Build history of the part. All positions in model axes, mm. A direction names the side the tool comes from. Round coordinates to 2 decimals unless told otherwise and drop trailing zeros. Write each loop counter-clockwise with the first axis right and the second up, starting at its lowest first coordinate (ties: lowest second). Pieces come first, ordered by that corner, then holes.
Item 1: Band-saw the part on B-B, the plane x = 65.5. Write the cut outline in (y, z) (3 decimals), then the cut area to 3 significant figures.
Item 2: Wall check: probe 1 along Y at (x, z) = (21, 83.5); probe 2 along X at (y, z) = (45.5, -12); probe 3 along Y at (x, z) = (14, 29). Give the ranges that are in metal, low to high.
Item 3: Band-saw the part on A-A, the plane z = 0. Write the cut outline in (x, y), then the cut area to 3 significant figures.
Item 4: Mould opens along Z. For faces 1 (the flat face through (7, 40, 127)), 2 (the flat face through (0, 63, 2)), 3 (the cylindrical face through (44.452, 4.056, 0.209)) say: +Z half, -Z half, draft (parallel to the pull), parting line (faces both ways), or undercut.
Item 5: 3-axis set-ups, long thin cutter, end or side, ignore diameter. For faces 4 (the flat face through (8, 71, 2)), 5 (the flat face through (7, 40, -127)), 6 (the flat face through (63, 4, -9.525)): which of +Z, -Z, +X, -X, +Y, -Y reach the whole face in a straight line?
Item 6: Band-saw the part on D-D, the plane y = 64. Write the cut outline in (x, z).
Item 7: Drop flat-ended pins along their axis: pin 1 Ø5 at (y, z) = (63, 40) entering from +X; pin 2 Ø4 at (x, z) = (54, 49.5) entering from +Y. Give the stop position or say it passes through.
Item 8: Band-saw the part on C-C, the plane z = -47. Write the cut outline in (x, y).
```python
from build123d import *

# Parameters (mm, degrees)
BOSS_EXTRUDE1_DEPTH = 127
CUT_EXTRUDE1_DEPTH  = 304.8


with BuildPart() as part:
    # Sketch1 → Boss-Extrude1 (new, symmetric)
    with BuildSketch(Plane.XY):
        with BuildLine():
            Line((0, 125), (0, 0))
            Line((0, 0), (125, 0))
            Line((125, 0), (125, 4))
            ThreePointArc((125, 4), (123.828427125, 6.828427125), (121, 8))
            Line((121, 8), (22, 8))
            ThreePointArc((22, 8), (12.100505063, 12.100505063), (8, 22))
            Line((8, 22), (8, 121))
            ThreePointArc((8, 121), (6.828427125, 123.828427125), (4, 125))
            Line((4, 125), (0, 125))
        make_face()
    extrude(amount=BOSS_EXTRUDE1_DEPTH, both=True)

    # Sketch2 → Cut-Extrude1 (cut)
    with BuildSketch(Plane(origin=(0, 8, 0), x_dir=(1, 0, 0), z_dir=(0, 1, 0))):
        with BuildLine():
            Line((53.975, 9.525), (73.025, 9.525))
            ThreePointArc((73.025, 9.525), (82.55, 0), (73.025, -9.525))
            Line((73.025, -9.525), (53.975, -9.525))
            ThreePointArc((53.975, -9.525), (44.45, 0), (53.975, 9.525))
        make_face()
    extrude(amount=-CUT_EXTRUDE1_DEPTH, mode=Mode.SUBTRACT)


solid = part.part
```
Results:
1. outline: (0, -127) - (8, -127) - (8, -9.525) - (0, -9.525) - close; (0, 9.525) - (8, 9.525) - (8, 127) - (0, 127) - close
1. area: 1,880 mm2
2. probe 1: y = 0 to 8.04
2. probe 2: x = 0 to 8
2. probe 3: y = 0 to 10.51
3. outline: (0, 0) - (44.45, 0) - (44.45, 8) - (22, 8) arc R14 cw to (8, 22) - (8, 121) arc R4 ccw to (4, 125) - (0, 125) - close; (82.55, 0) - (125, 0) - (125, 4) arc R4 ccw to (121, 8) - (82.55, 8) - close
3. area: 1,670 mm2
4. face 1: +Z half
4. face 2: draft
4. face 3: undercut
5. face 4: +Z, -Z, +X, +Y
5. face 5: -Z, +X, -X, +Y, -Y
5. face 6: +Y, -Y
6. outline: (0, -127) - (8, -127) - (8, 127) - (0, 127) - close
7. pin 1: stops at x = 8
7. pin 2: stops at y = 8
8. outline: (0, 0) - (125, 0) - (125, 4) arc R4 ccw to (121, 8) - (22, 8) arc R14 cw to (8, 22) - (8, 121) arc R4 ccw to (4, 125) - (0, 125) - close
